Can you work these out from the drawing? Everything is in mm from the part's minimum corner. Coordinates: 2 decimals unless noted, no trailing zeros. Write each loop counter-clockwise with the first axis right and the second up, starting at its lowest first coordinate (ties: lowest second). Pieces come first, ordered by that corner, then holes. Notation, with made-up numbers: (11.5, -16.5) - (50.5, -16.5) arc R19 ccw to (50.5, -3.5) - close; hole circle Ø2 at (30.5, -7). An arc over 180 degrees is marked (long way). One line per question, with ' | ' between items. Start each with the question number.
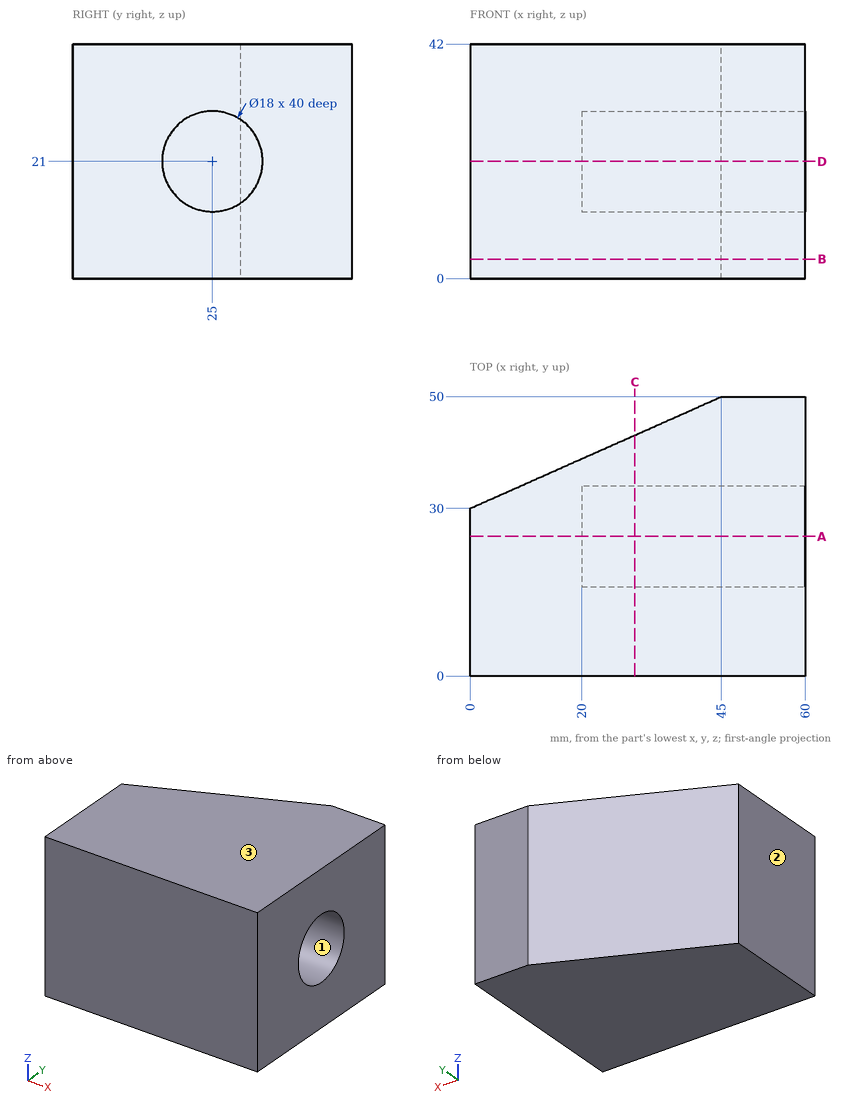
(1) If we section it at D-D on z = 21: List the corners of the cut face in (x, y) for me.
(2) If I drill on probe 1 along Z at (x, y) = (38, 25); probe 2 along X at (y, z) = (22, 21); probe 3 along Z at (x, y) = (38.5, 19), over which ranges is the centre line in solid material (lowest first)?
(3) If we section it at B-B on z = 3.5: List the corners of the cut face in (x, y) for me.
(4) If we section it at A-A on y = 25: List the corners of the cut face in (x, z) for me, plus the area to 3 significant figures.
(5) I'm going to push flat-ended pins straight in: pin 1 (1.5 mm diameter, centred on x = 17, z = 29, fed in from +Y); pin 2 (10 mm diameter, centred on x = 51, y = 28, fed in from -Z). Where does each tip first touch, or does it pass through?
(6) If we section it at C-C on x = 29.5: List the corners of the cut face in (y, z) for me, plus the area to 3 significant figures.
(7) If we mould it in two halves opening along Z, with no side actions, what happens to the marked faces 1, 2 and 3? For each: +Z half, -Z half, draft (parallel to the pull), parting line (faces both ways), or undercut.
Values:
1) outline: (0, 0) - (60, 0) - (60, 16) - (20, 16) - (20, 34) - (60, 34) - (60, 50) - (45, 50) - (0, 30) - close
2) probe 1: 0 to 12, 30 to 42 | probe 2: 0 to 20 | probe 3: 0 to 14.29, 27.71 to 42
3) outline: (0, 0) - (60, 0) - (60, 50) - (45, 50) - (0, 30) - close
4) outline: (0, 0) - (60, 0) - (60, 12) - (20, 12) - (20, 30) - (60, 30) - (60, 42) - (0, 42) - close | area: 1,800 mm2
5) pin 1: y = 37.89 | pin 2: z = 0
6) outline: (0, 0) - (43.11, 0) - (43.11, 42) - (0, 42) - close; hole circle Ø18 at (25, 21) | area: 1,560 mm2
7) face 1: undercut | face 2: draft | face 3: +Z half
